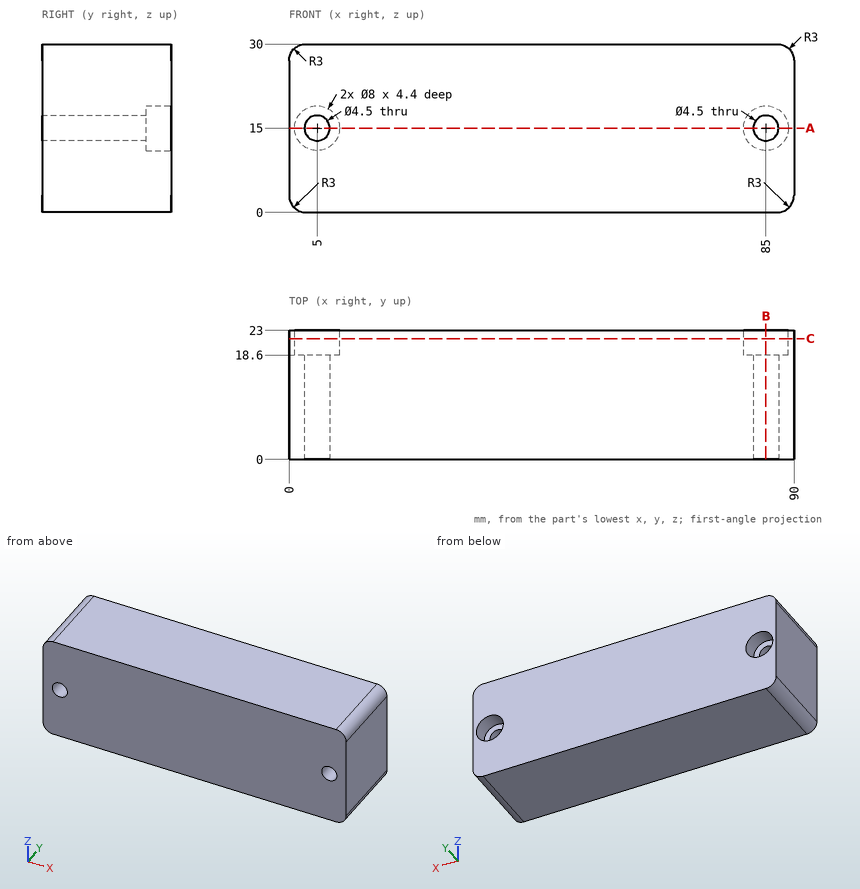
Design review of the part shown in the three views and the two pictorial views. Dimensions are in mm from the part's minimum x, y and z. Give positions to 0.01 mm unless a question says otherwise; leave off trailing zeros. Loops run counter-clockwise (first coordinate to the right, second up) from the corner with the lowest first, then second, coordinate; pieces in that order, holes last. Notation, with made-up numbers: (-31, 84) -> (5, 84) arc R19 ccw to (5, 101) -> close; hole circle Ø8 at (-11.5, -21.5). An arc over 180 degrees is marked (long way). Put each result on its own line as item: value. Start each with the question number.
1. We need section C-C on y = 21.5. State the section outline as (x, z) points.
2. We need section B-B on x = 85. State the section outline as (y, z) points.
3. Clearance check with flat-ended pins moving along their axes: P1, Ø3.5, axis at x = 5, z = 15, coming from the -Y side; P2, Ø6, axis at x = 85, z = 15, coming from the +Y side. State where each tip first meets the part, or that it passes through.
4. We need section A-A on z = 15. State the section outline as (x, y) points, then the cut area to 3 significant figures.
5. Wall thickness on probe 1 along X at (y, z) = (11.5, 15); probe 2 along Z at (x, y) = (5, 21.9); probe 3 along Z at (x, y) = (85, 14.75): over which ranges is each line inside the solid? List them lowest first.
Determined:
1. outline: (0, 3) arc R3 ccw to (3, 0) -> (87, 0) arc R3 ccw to (90, 3) -> (90, 27) arc R3 ccw to (87, 30) -> (3, 30) arc R3 ccw to (0, 27) -> close; hole circle Ø8 at (5, 15); hole circle Ø8 at (85, 15)
2. outline: (0, 0) -> (23, 0) -> (23, 11) -> (18.6, 11) -> (18.6, 12.75) -> (0, 12.75) -> close; (0, 17.25) -> (18.6, 17.25) -> (18.6, 19) -> (23, 19) -> (23, 30) -> (0, 30) -> close
3. P1: through
3. P2: y = 18.6
4. outline: (0, 0) -> (2.75, 0) -> (2.75, 18.6) -> (1, 18.6) -> (1, 23) -> (0, 23) -> close; (7.25, 0) -> (82.75, 0) -> (82.75, 18.6) -> (81, 18.6) -> (81, 23) -> (9, 23) -> (9, 18.6) -> (7.25, 18.6) -> close; (87.25, 0) -> (90, 0) -> (90, 23) -> (89, 23) -> (89, 18.6) -> (87.25, 18.6) -> close
4. area: 1,830 mm^2
5. probe 1: 0 to 2.75, 7.25 to 82.75, 87.25 to 90
5. probe 2: 0 to 11, 19 to 30
5. probe 3: 0 to 12.75, 17.25 to 30
